Read the model definition and answer for the solid it produces. Units are mm, in the model's axes. Give positions to 0.01 mm unless a question says otherwise; leave off trailing zeros. Write each loop counter-clockwise with the first axis right and the second up, starting at its lowest first coordinate (ties: lowest second). Pieces come first, ordered by that corner, then holes. Notation, with made-up numbers: M 2,39 L 30,39 A15 cw 30,51 Z; hole C 21.25,0.5 d5. An arc over 180 degrees is marked long. Put each result on its own line as item: value.
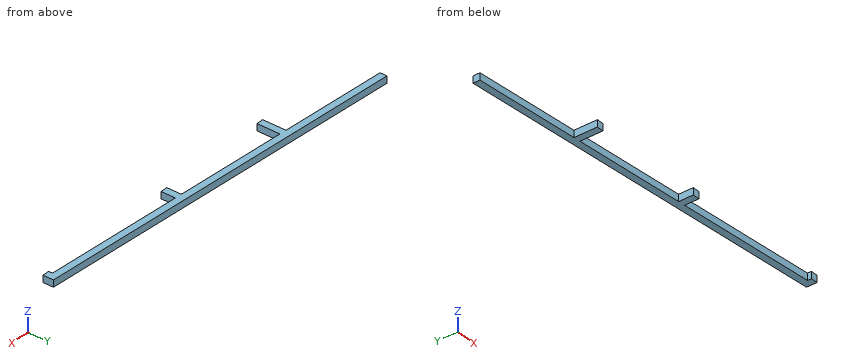
from build123d import *

# Parameters (mm, degrees)
BOSS_EXTRUDE1_DEPTH = 40


with BuildPart() as part:
    # Sketch1 → Boss-Extrude1 (new body)
    with BuildSketch(Plane.XY):
        Polygon((2200, 0), (2200, 60), (0, 220), (0, 179.894354388), (620, 134.803445298), (620, 0), (660, 0), (660, 131.894354388), (1310, 84.621627116), (1310, 0), (1350, 0), (1350, 81.712536207), (2160, 22.803445298), (2160, 0), align=None)
    extrude(amount=BOSS_EXTRUDE1_DEPTH)


solid = part.part
(1) Section B-B on x = 186 is taken. Determine the outline of the cut face in (y, z).
Result:
outline: M 166.37,0 L 206.47,0 L 206.47,40 L 166.37,40 Z
(2) Section A-A on z = 7 is taken. Determine the outline of the cut face in (x, y).
Result:
outline: M 0,179.89 L 620,134.8 L 620,0 L 660,0 L 660,131.89 L 1310,84.62 L 1310,0 L 1350,0 L 1350,81.71 L 2160,22.8 L 2160,0 L 2200,0 L 2200,60 L 0,220 Z
(3) Given pin 1 Ø12 at (y, z) = (25, 24) entering from -X; pin 2 Ø1.5 at (x, z) = (770.5, 14) entering from +Y; pin 3 Ø2 at (x, z) = (1584.5, 24.5) entering from -Y, each flat-ended and moving along its own axis, determine where each tip first touches the part or whether it passes through.
Result:
pin 1: stops at x = 620
pin 2: stops at y = 164.02
pin 3: stops at y = 64.59
(4) Straight lines are drawn through the part: line 1 along Y through (x, z) = (1225, 28); line 2 along Y through (x, z) = (2083.5, 4.5). For each, find the intervals that lie inside material, in ascending order. Write a range as from..to.
Result:
line 1: y = 90.8..130.91
line 2: y = 28.37..68.47
